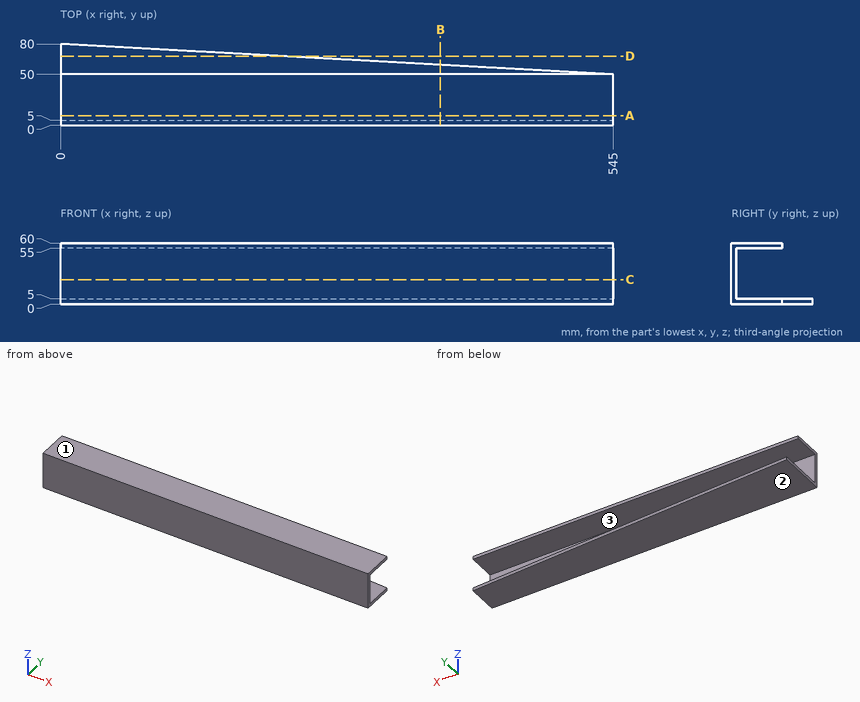
Geometry check sheet. Reference: drawing and pictorial views, mm from the part's lowest x, y, z. Give positions to 0.01 mm unless a question says otherwise; leave off trailing zeros. Order: outer loops, then holes, each group sorted by start corner. A loop starts at its lowest first (then second) coordinate and runs counter-clockwise, first axis right, second up. Notation, with made-up numbers: M -18,-2 L 0,-2 A21 ccw 0,14 Z; hole C 46.25,-32 d8. An arc over 180 degrees is marked long. Answer in a Markdown table with one row per item.
1) Cross-section at C-C, the plane z = 24. Enter the section's corners in (x, y).
Filled sheet:
| item | result |
|---|---|
| outline | M 0,0 L 545,0 L 545,5 L 0,5 Z |
2) Cross-section at B-B, the plane x = 374.5. Enter the section's corners in (y, z).
Filled sheet:
| item | result |
|---|---|
| outline | M 0,0 L 59.39,0 L 59.39,5 L 5,5 L 5,55 L 50,55 L 50,60 L 0,60 Z |
3) Release check for a two-part mould opening along Z. For the marked faces 1, 2 and 3 record: +Z half, -Z half, draft (parallel to the pull), parting line (faces both ways), or undercut.
Filled sheet:
| item | result |
|---|---|
| face 1 | +Z half |
| face 2 | -Z half |
| face 3 | undercut |
4) Gauge pin test, flat ends, axial feed: P1, Ø1.5, axis at x = 143, z = 57.5, coming from the +Y side; P2, Ø12, axis at y = 15, z = 24.5, coming from the +X side; P3, Ø5, axis at x = 197, z = 21, coming from the +Y side. Record the tip position at first contact, or that the pin passes through.
Filled sheet:
| item | result |
|---|---|
| P1 | stops at y = 50 |
| P2 | passes through |
| P3 | stops at y = 5 |
5) Cross-section at D-D, the plane y = 68. Enter the section's corners in (x, z), plus the area to 3 significant figures.
Filled sheet:
| item | result |
|---|---|
| outline | M 0,0 L 218,0 L 218,5 L 0,5 Z |
| area | 1,090 mm2 |
6) Thickness scan on L1, parallel to Z at x = 431, y = 11; L2, parallel to Z at x = 396.5, y = 53.5. Record the ranges inside material, lowest first. Write a range as [from, to].
Filled sheet:
| item | result |
|---|---|
| L1 | z = [0, 5], [55, 60] |
| L2 | z = [0, 5] |
7) Cross-section at A-A, the plane y = 9.5. Enter the section's corners in (x, z), plus the area to 3 significant figures.
Filled sheet:
| item | result |
|---|---|
| outline | M 0,0 L 545,0 L 545,5 L 0,5 Z; M 0,55 L 545,55 L 545,60 L 0,60 Z |
| area | 5,450 mm2 |
